Source: three-view drawing plus pictorial views. Frame: mm from the lowest corner of the part. A direction names the side the tool comes from. Coordinates: 2 decimals unless noted, no trailing zeros. Write each loop counter-clockwise with the first axis right and the second up, starting at its lowest first coordinate (ties: lowest second). Pieces come first, ordered by that corner, then holes. Notation, with made-up numbers: (59.5, 89) - (65.5, 89) arc R13 ccw to (65.5, 102) - close; hole circle Ø7 at (-24, 54). An arc over 180 degrees is marked (long way). Put each result on its own line as item: value.
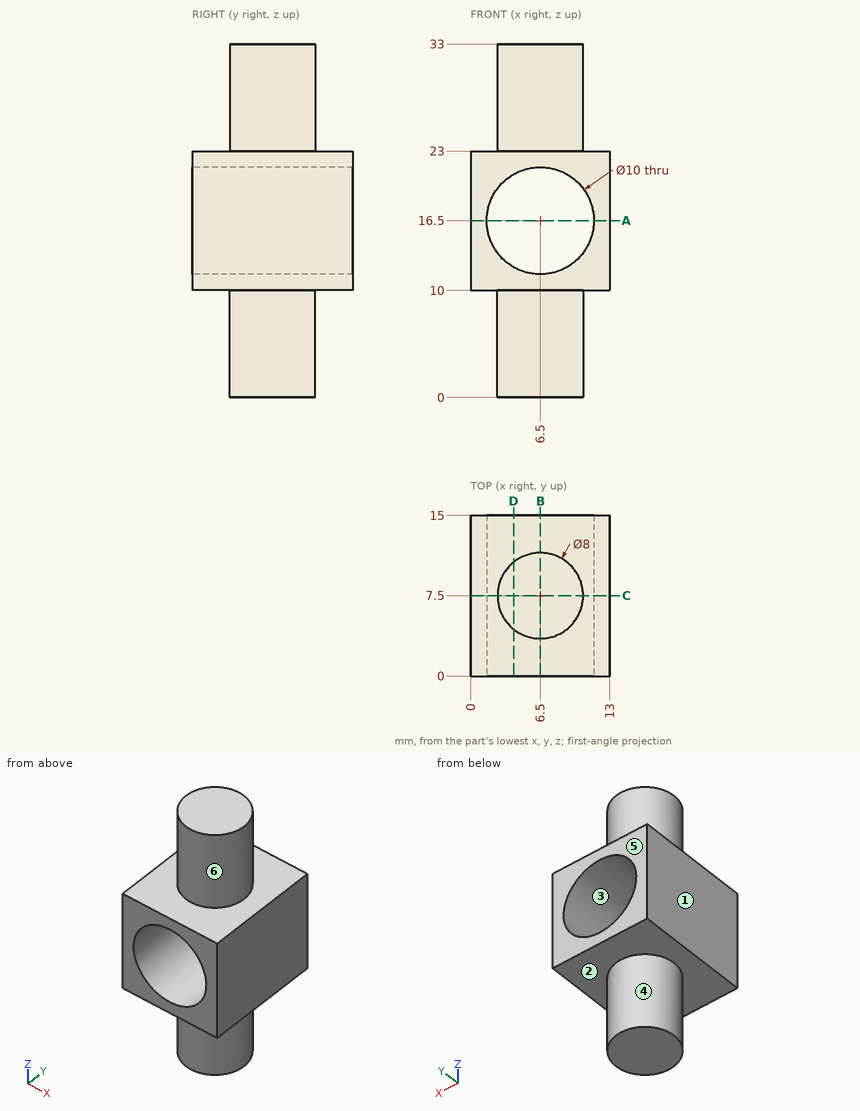
1. Section query A-A (z = 16.5). Return loops of the section in (x, y).
Answer below:
outline: (0, 0) - (1.5, 0) - (1.5, 15) - (0, 15) - close; (11.5, 0) - (13, 0) - (13, 15) - (11.5, 15) - close
2. Section query D-D (x = 4). Return loops of the section in (y, z).
Answer below:
outline: (0, 10) - (4.38, 10) - (4.38, 0) - (10.62, 0) - (10.62, 10) - (15, 10) - (15, 12.17) - (0, 12.17) - close; (0, 20.83) - (15, 20.83) - (15, 23) - (10.62, 23) - (10.62, 33) - (4.38, 33) - (4.38, 23) - (0, 23) - close
3. Section query B-B (x = 6.5). Return loops of the section in (y, z).
Answer below:
outline: (0, 10) - (3.5, 10) - (3.5, 0) - (11.5, 0) - (11.5, 10) - (15, 10) - (15, 11.5) - (0, 11.5) - close; (0, 21.5) - (15, 21.5) - (15, 23) - (11.5, 23) - (11.5, 33) - (3.5, 33) - (3.5, 23) - (0, 23) - close
4. Pin query (flat end, axial travel): pin 1 Ø2 at (x, y) = (8, 2) entering from -Z. Return the tip coordinate at first contact, or that it passes through.
Answer below:
pin 1: stops at z = 10
5. Ray query, probe 1 along X at (y, z) = (5.5, 16.5); probe 2 along Z at (x, y) = (7, 4.5); probe 3 along Z at (x, y) = (1, 3.25). Return the intervals inside material, ascending. Write a range as from..to.
Answer below:
probe 1: x = 0..1.5, 11.5..13
probe 2: z = 0..11.53, 21.47..33
probe 3: z = 10..23
6. Mould query, pull axis X, two halves, no side actions, for the marked faces 1, 2, 3 and 4. Classes: +X half, -X half, draft (parallel to the pull), parting line (faces both ways), or undercut.
Answer below:
face 1: -X half
face 2: draft
face 3: undercut
face 4: parting line
7. Set-up query: the marked faces 5 and 6. Return all of +Z, -Z, +X, -X, +Y, -Y with unobstructed straight access to the full face (end or side cutting, diameter ignored); none if empty.
Answer below:
face 5: +Z, -Z, +X, -X, +Y
face 6: +Z
8. Section query C-C (y = 7.5). Return loops of the section in (x, z).
Answer below:
outline: (0, 10) - (2.5, 10) - (2.5, 0) - (10.5, 0) - (10.5, 10) - (13, 10) - (13, 23) - (10.5, 23) - (10.5, 33) - (2.5, 33) - (2.5, 23) - (0, 23) - close; hole circle Ø10 at (6.5, 16.5)
